Here's the drawing with two shaded views (mm, measured from the low corner). I have some questions. A direction names the side the tool comes from. Coordinates: 2 decimals unless noted, no trailing zeros. Write each loop counter-clockwise with the first axis right and the second up, starting at its lowest first coordinate (ties: lowest second). Pieces come first, ordered by that corner, then holes.
Item 1: If I drill on probe 1 along Z at (x, y) = (3.35, 3.65) (1 decimal); probe 2 along Y at (x, z) = (1.55, 8.75) (1 decimal); probe 3 along Z at (x, y) = (0.7, 2.9), over which ranges is the centre line in solid material (lowest first)?
Item 2: I want a section at B-B on z = 3.25. Please give me the cut outline in (x, y).
Item 3: Which directions (+Z, -Z, +X, -X, +Y, -Y) give clear straight access to the entire face, cutting with the end or side of a thin tool? Please do the marked faces 5 and 6.
Item 4: Thinking about a two-plate mould opening in Y: for the marked faces 1, 2, 3 and 4, which applies, +Y half, -Y half, draft (parallel to the pull), parting line (faces both ways), or undercut?
Item 5: I want a section at A-A on z = 8.5. Please give me the cut outline in (x, y).
Item 6: For P1, Ø1, axis at x = 4.5, y = 2, coming from the -Z side (1 decimal); P2, Ø1.5, axis at y = 3.5, z = 1.5, coming from the +X side, each with a flat end and sliding along its axis, tell me the tip position at first contact or that it passes through.
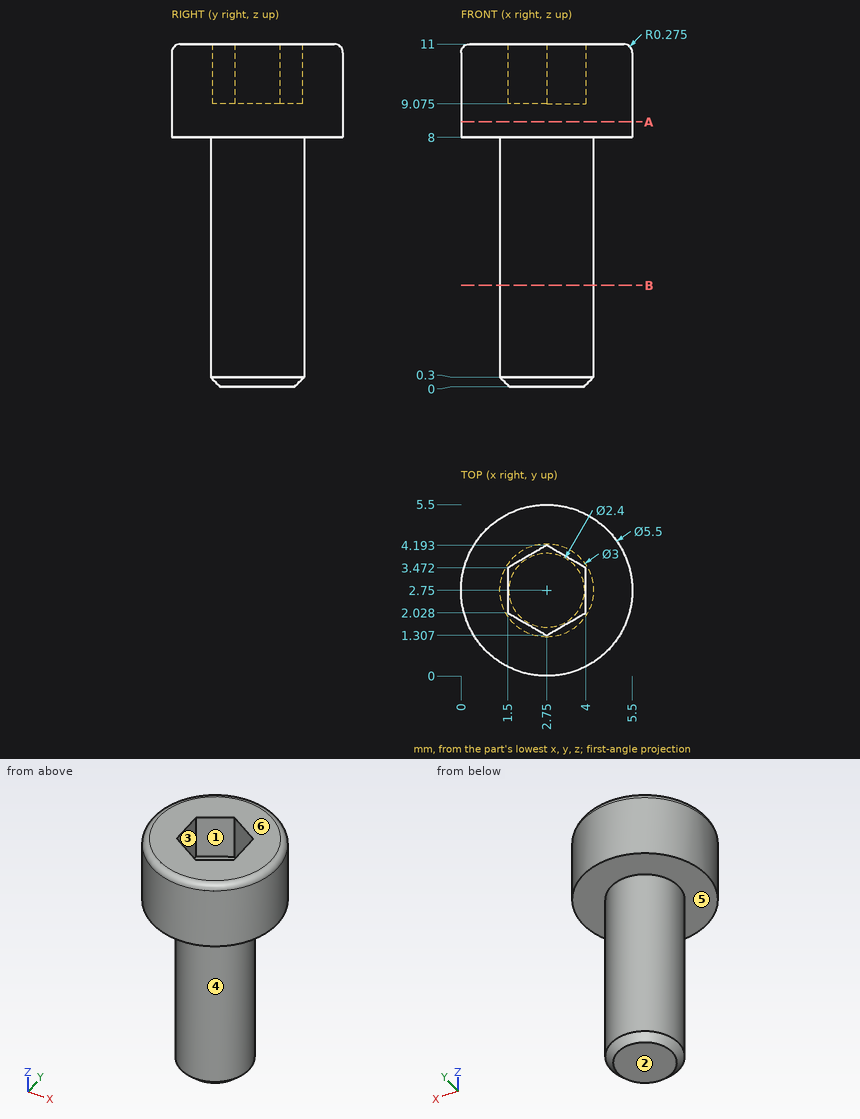
Response values:
1. probe 1: z = 0 to 9.1
1. probe 2: y = 0.3 to 5.2
1. probe 3: z = 8 to 11
2. outline: circle Ø3 at (2.75, 2.75)
3. face 5: -Z
3. face 6: +Z, +X, -X, +Y, -Y
4. face 1: undercut
4. face 2: draft
4. face 3: undercut
4. face 4: parting line
5. outline: circle Ø5.5 at (2.75, 2.75)
6. P1: stops at z = 0.2
6. P2: stops at x = 4.25
